Can you work these out from the model? Positions are in its coordinate system, mm. Round coordinates to 2 decimals unless told otherwise and drop trailing zeros. Write each loop counter-clockwise with the first axis right and the second up, starting at its lowest first coordinate (ties: lowest second). Pieces come first, ordered by that corner, then holes. Notation, with made-up numbers: (41, 12) -> (71, 12) arc R9 cw to (71, 17) -> close; hole circle Ø6 at (15.5, 55). An arc over 180 degrees is marked (long way). Write item = value, one per line. Start each with the question number.
1) I'm going to push flat-ended pins straight in: pin 1 (2.5 mm diameter, centred on y = 76.5, z = 2.5, fed in from +X); pin 2 (1.5 mm diameter, centred on x = 73, z = 3, fed in from -Y); pin 3 (2.5 mm diameter, centred on y = 2, z = 3.5, fed in from -X); pin 4 (6 mm diameter, centred on x = 19, y = 54, fed in from -Z). Where does each tip first touch, or does it pass through?
2) If I drill on line 1 (Y direction, x = 61, z = 2.7); line 2 (X direction, y = 38, z = 4.6); line 3 (Y direction, x = 68.5, z = 2.15), over which ranges is the centre line in solid material (lowest first)?
3) Imagine slicing it at C-C, the plane y = 34. Please give me the cut outline in (x, z), then the cut area to 3 significant figures.
4) Imagine slicing it at A-A, the plane x = 9.5. Please give me the cut outline in (y, z).
5) Imagine slicing it at B-B, the plane z = 1.5. Please give me the cut outline in (x, y).
from build123d import *

# Parameters (mm, degrees)
EXTRUDE_1_DEPTH     = 5
CUT_EXTRUDE_2_DEPTH = 5


with BuildPart() as part:
    # 草图1 → 凸台-拉伸1 (new body)
    with BuildSketch(Plane.XY):
        Polygon((12, 0), (27, 0), (27, 5), (52, 5), (52, 0), (67, 0), (67, 5), (79, 5), (79, 72.9), (67, 72.9), (67, 77.9), (52, 77.9), (52, 72.9), (27, 72.9), (27, 77.9), (12, 77.9), (12, 72.9), (0, 72.9), (0, 5), (12, 5), align=None)
    extrude(amount=EXTRUDE_1_DEPTH)

    # 草图2 → 切除-拉伸2 (cut)
    with BuildSketch(Plane(origin=(0, 0, 0), x_dir=(-1, 0, 0), z_dir=(0, 0, -1))):
        with BuildLine():
            Line((-70.163147459, 44.470964867), (-7.979563682, 44.470964867))
            ThreePointArc((-7.979563682, 44.470964867), (-1.539904649, 38.031305835), (-7.979563682, 31.591646802))
            Line((-7.979563682, 31.591646802), (-70.163147459, 31.591646802))
            ThreePointArc((-70.163147459, 31.591646802), (-76.602806492, 38.031305835), (-70.163147459, 44.470964867))
        make_face()
    extrude(amount=-CUT_EXTRUDE_2_DEPTH, mode=Mode.SUBTRACT)


solid = part.part
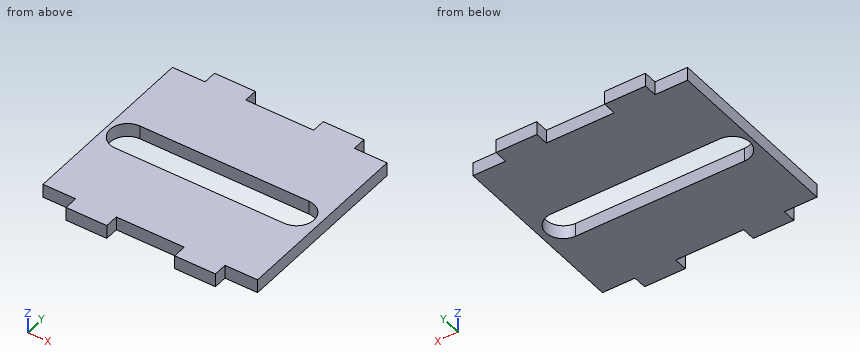
Reported:
q1.pin_1 = 67
q1.pin_2 = 5
q1.pin_3 = 12
q1.pin_4 = 0
q2.line_1 = 0 to 31.59, 44.47 to 77.9
q2.line_2 = 0 to 1.54, 76.6 to 79
q2.line_3 = 5 to 31.59, 44.47 to 72.9
q3.outline = (0, 0) -> (2.96, 0) -> (2.96, 5) -> (0, 5) -> close; (75.18, 0) -> (79, 0) -> (79, 5) -> (75.18, 5) -> close
q3.area = 33.9 mm²
q4.outline = (5, 0) -> (31.59, 0) -> (31.59, 5) -> (5, 5) -> close; (44.47, 0) -> (72.9, 0) -> (72.9, 5) -> (44.47, 5) -> close
q5.outline = (0, 5) -> (12, 5) -> (12, 0) -> (27, 0) -> (27, 5) -> (52, 5) -> (52, 0) -> (67, 0) -> (67, 5) -> (79, 5) -> (79, 72.9) -> (67, 72.9) -> (67, 77.9) -> (52, 77.9) -> (52, 72.9) -> (27, 72.9) -> (27, 77.9) -> (12, 77.9) -> (12, 72.9) -> (0, 72.9) -> close; hole (7.98, 31.59) -> (70.16, 31.59) arc R6.44 ccw to (70.16, 44.47) -> (7.98, 44.47) arc R6.44 ccw to start
